Could you check a few things on this drawing? It's one solid part, dimensions in mm from its lowest x, y, z. A direction names the side the tool comes from. Give positions to 0.01 mm unless a question says otherwise; leave off trailing zeros. Loops run counter-clockwise (first coordinate to the right, second up) from the corner with the lowest first, then second, coordinate; pieces in that order, holes last. Notation, with made-up numbers: (65, -13) - (110, -13) arc R8 cw to (110, -4) - close; hole circle Ø2 at (-35.5, 82). An arc over 180 degrees is marked (long way). Answer as a JSON object with one key per item and string values.
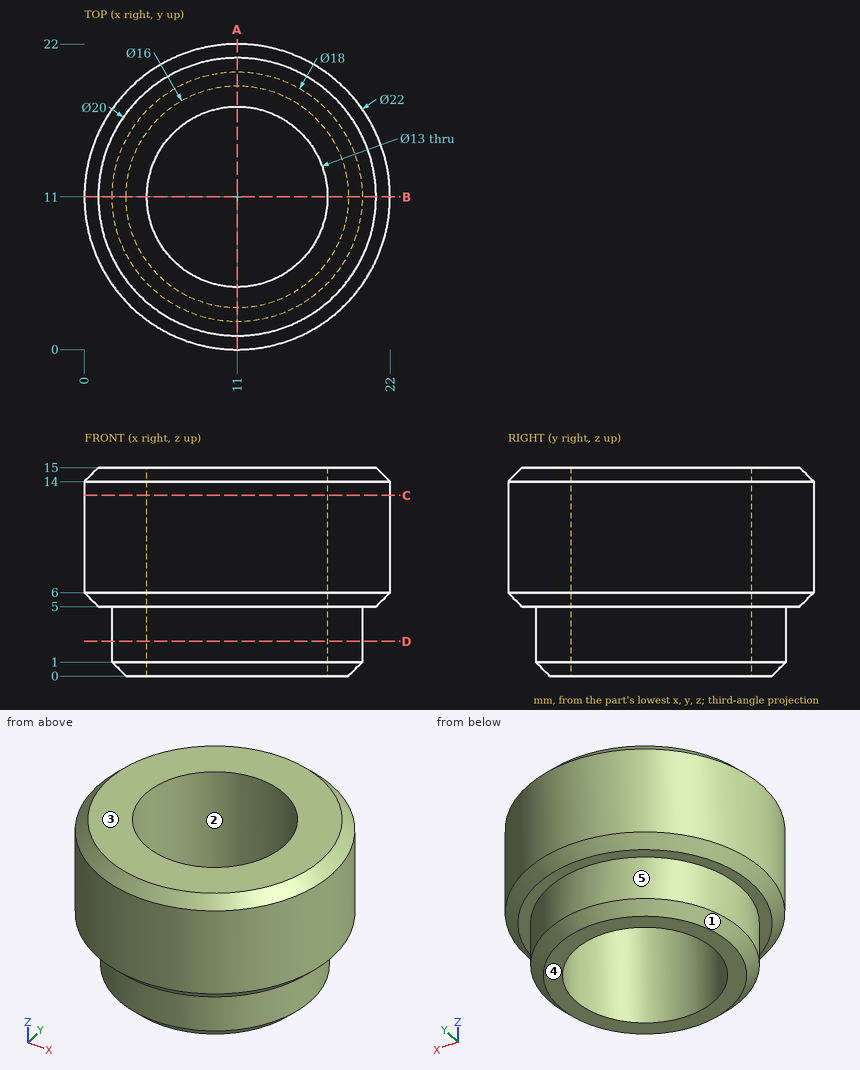
1) Which directions (+Z, -Z, +X, -X, +Y, -Y) give clear straight access to the entire face, cutting with the end or side of a thin tool? Please do the marked faces 4 and 5.
Check sheet entries:
{"face 4": "-Z, +X, -X, +Y, -Y", "face 5": "-Z"}
2) Imagine slicing it at A-A on x = 11. Write out the boundary of the cut face in (y, z).
Check sheet entries:
{"outline": "(0, 6) - (1, 5) - (2, 5) - (2, 1) - (3, 0) - (4.5, 0) - (4.5, 15) - (1, 15) - (0, 14) - close; (17.5, 0) - (19, 0) - (20, 1) - (20, 5) - (21, 5) - (22, 6) - (22, 14) - (21, 15) - (17.5, 15) - close"}
3) Imagine slicing it at D-D on z = 2.5. Write out the boundary of the cut face in (x, y), and give its area (3 significant figures).
Check sheet entries:
{"outline": "circle Ø18 at (11, 11); hole circle Ø13 at (11, 11)", "area": "122 mm2"}
4) I'm going to push flat-ended pins straight in: P1, Ø4, axis at x = 18.5, z = 12.5, coming from the -Y side; P2, Ø5, axis at x = 8, z = 8.5, coming from the +Y side; P3, Ø6, axis at y = 16.5, z = 11.5, coming from the +X side. Where does each tip first touch, or does it pass through?
Check sheet entries:
{"P1": "y = 1.47", "P2": "y = 21.99", "P3": "x = 21.71"}
5) If we mould it in two halves opening along Y, with no side actions, what happens to the marked faces 1, 2 and 3? For each: released by +Y, released by -Y, zero draft, split by the parting line, or undercut.
Check sheet entries:
{"face 1": "split by the parting line", "face 2": "undercut", "face 3": "zero draft"}
6) I need wall thicknesses on L1, parallel to Y at x = 11, z = 4.75; L2, parallel to Y at x = 11, z = 11.75; L3, parallel to X at y = 10, z = 14.5. Which ranges of each line are inside material? Lowest first, please.
Check sheet entries:
{"L1": "2 to 4.5, 17.5 to 20", "L2": "0 to 4.5, 17.5 to 22", "L3": "0.55 to 4.58, 17.42 to 21.45"}
7) Imagine slicing it at C-C on z = 13. Write out the boundary of the cut face in (x, y).
Check sheet entries:
{"outline": "circle Ø22 at (11, 11); hole circle Ø13 at (11, 11)"}
